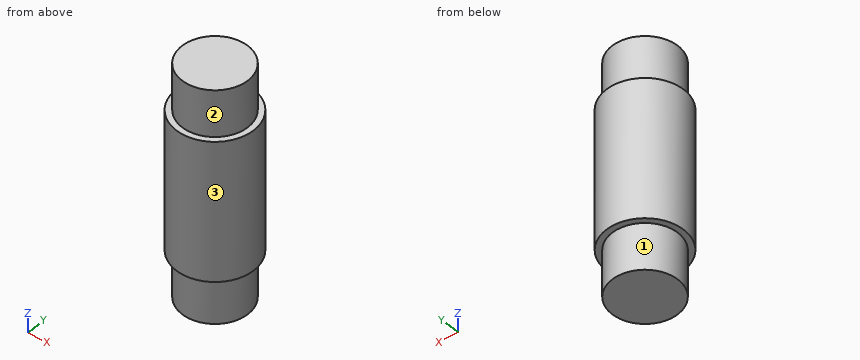
```python
from build123d import *

# Parameters (mm, degrees)
SKETCH_1_R      = 10
EXTRUDE_1_DEPTH = 18
SKETCH_2_R      = 8.5
EXTRUDE_2_DEPTH = 12


with BuildPart() as part:
    # 草图1 → 凸台-拉伸1 (new, symmetric)
    with BuildSketch(Plane.XY):
        Circle(SKETCH_1_R)
    extrude(amount=EXTRUDE_1_DEPTH, both=True)

    # 草图2 → 凸台-拉伸2 (add)
    with BuildSketch(Plane.XY.offset(18)):
        Circle(SKETCH_2_R)
    extrude_2 = extrude(amount=EXTRUDE_2_DEPTH)

    # 镜向1: 凸台-拉伸2 across plane
    add(extrude_2.mirror(Plane.XY))


solid = part.part
```
Input: part model. Units: mm. Frame: model coordinates. Face numbers are marked on the shaded views. A direction names the side the tool comes from. Coordinates: 2 decimals unless noted, no trailing zeros. Write each loop counter-clockwise with the first axis right and the second up, starting at its lowest first coordinate (ties: lowest second). Pieces come first, ordered by that corner, then holes.
1) Pin query (flat end, axial travel): pin 1 Ø10 at (x, y) = (-5, -7.5) entering from -Z; pin 2 Ø4 at (x, z) = (7.5, 0) entering from -Y; pin 3 Ø3 at (y, z) = (-7, -3.5) entering from +X; pin 4 Ø10 at (x, z) = (-7.5, -13) entering from +Y. Return the tip coordinate at first contact, or that it passes through.
2) Set-up query: the marked faces 1, 2 and 3. Return all of +Z, -Z, +X, -X, +Y, -Y with unobstructed straight access to the full face (end or side cutting, diameter ignored); none if empty.
3) Section C-C on z = -12. Output: boundary loops of the cut face in (x, y), and give its area (3 significant figures).
4) Material intervals for line 1 along Z through (x, y) = (-5, -8.5); line 2 along Y through (x, z) = (-5.25, 2.5); line 3 along X through (y, z) = (-0.25, 6), sorted ascending.
5) Section A-A on x = 0. Output: boundary loops of the cut face in (y, z), and give its area (3 significant figures).
Check result:
1. pin 1: stops at z = -30
1. pin 2: stops at y = -8.35
1. pin 3: stops at x = 8.35
1. pin 4: stops at y = 9.68
2. face 1: -Z
2. face 2: +Z
2. face 3: +Z, -Z
3. outline: circle Ø20 at (0, 0)
3. area: 314 mm2
4. line 1: z = -18 to 18
4. line 2: y = -8.51 to 8.51
4. line 3: x = -10 to 10
5. outline: (-10, -18) - (-8.5, -18) - (-8.5, -30) - (8.5, -30) - (8.5, -18) - (10, -18) - (10, 18) - (8.5, 18) - (8.5, 30) - (-8.5, 30) - (-8.5, 18) - (-10, 18) - close
5. area: 1,130 mm2
